Source: three-view drawing plus pictorial views. Frame: mm from the lowest corner of the part. Round coordinates to 2 decimals unless told otherwise and drop trailing zeros. Write each loop counter-clockwise with the first axis right and the second up, starting at its lowest first coordinate (ties: lowest second). Pieces come first, ordered by that corner, then holes. Notation, with made-up numbers: (38.5, 81) - (70.5, 81) arc R32 cw to (70.5, 118) - close; hole circle Ø8 at (-2, 47.25). An arc over 180 degrees is marked (long way). Write each question's results on one line, items separated by ' | '.
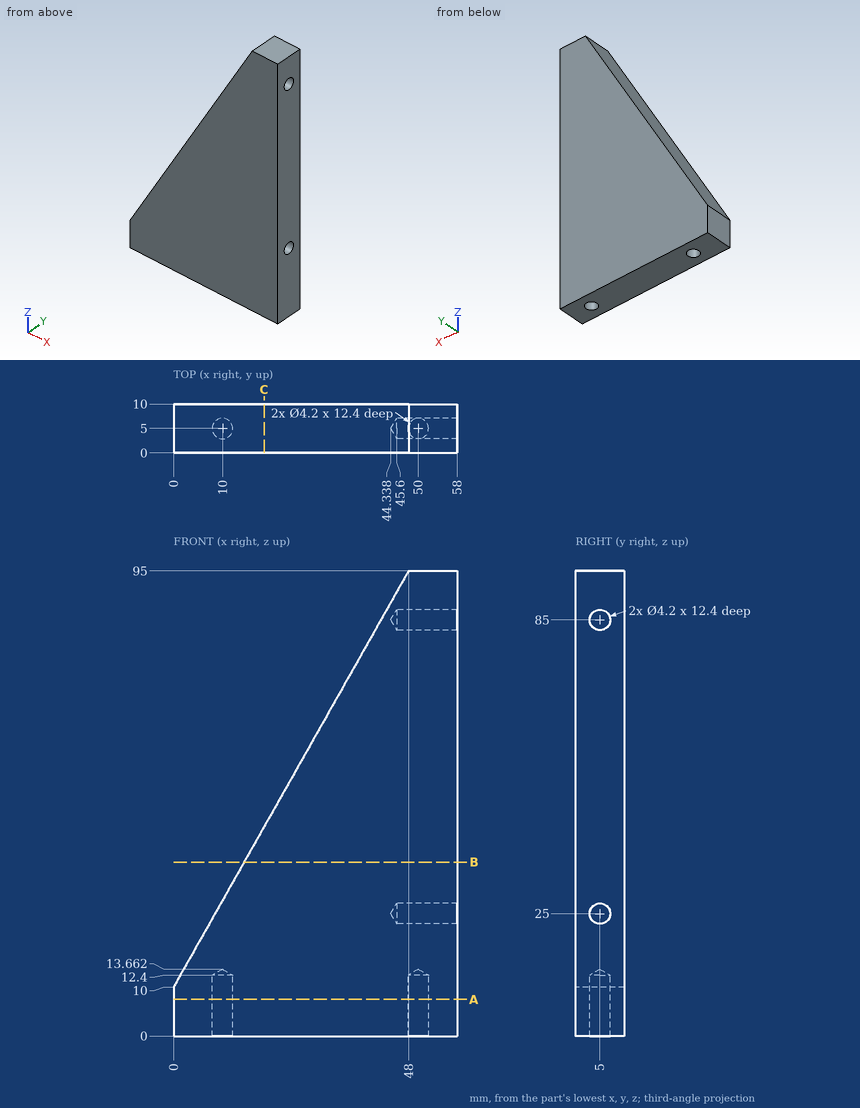
Q1. Ray query, line 1 along X through (y, z) = (5, 3.25); line 2 along Z through (x, y) = (55, 5); line 3 along Y through (x, z) = (52.25, 25). Return the intervals inside material, ascending.
Answer block:
line 1: 0 to 7.9, 12.1 to 47.9, 52.1 to 58 | line 2: 0 to 22.9, 27.1 to 82.9, 87.1 to 95 | line 3: 0 to 2.9, 7.1 to 10
Q2. Section query A-A, the plane z = 7.5. Return loops of the section in (x, y), plus the area to 3 significant figures.
Answer block:
outline: (0, 0) - (58, 0) - (58, 10) - (0, 10) - close; hole circle Ø4.2 at (10, 5); hole circle Ø4.2 at (50, 5) | area: 552 mm2
Q3. Pin query (flat end, axial travel): pin 1 (4 mm diameter, centred on x = 40.5, y = 3, fed in from +Z); pin 2 (4 mm diameter, centred on y = 5.5, z = 14.5, fed in from -X); pin 3 (3.5 mm diameter, centred on x = 10, y = 5, fed in from +Z). Return the tip coordinate at first contact, or that it passes through.
Answer block:
pin 1: z = 85.26 | pin 2: x = 1.41 | pin 3: z = 30.81
Q4. Section query B-B, the plane z = 35.5. Return loops of the section in (x, y).
Answer block:
outline: (14.4, 0) - (58, 0) - (58, 10) - (14.4, 10) - close
Q5. Section query C-C, the plane x = 18.5. Return loops of the section in (y, z), plus the area to 3 significant figures.
Answer block:
outline: (0, 0) - (10, 0) - (10, 42.76) - (0, 42.76) - close | area: 428 mm2
